from build123d import *

# Parameters (mm, degrees)
BOSS_EXTRUDE1_DEPTH = 580
BOSS_EXTRUDE2_DEPTH = 472
BOSS_EXTRUDE3_DEPTH = 580


with BuildPart() as part:
    # Sketch1 → Boss-Extrude1 (new body)
    with BuildSketch(Plane.XY):
        Polygon((-10.73531847, 12.748914521), (-45.73531847, 12.748914521), (-45.73531847, -37.251085479), (-10.73531847, -37.251085479), (-10.73531847, -33.251085479), (-41.73531847, -33.251085479), (-41.73531847, 8.748914521), (-10.73531847, 8.748914521), align=None)
    extrude(amount=BOSS_EXTRUDE1_DEPTH)

    # Sketch2 → Boss-Extrude2 (add)
    with BuildSketch(Plane(origin=(-41.73531847, 0, 0), x_dir=(0, 0, -1), z_dir=(1, 0, 0))):
        Polygon((-545, 12.748914521), (-580, 12.748914521), (-580, -37.251085479), (-545, -37.251085479), (-545, -33.251085479), (-576, -33.251085479), (-576, 8.748914521), (-545, 8.748914521), align=None)
        Polygon((-35, -33.251085479), (-35, -37.251085479), (0, -37.251085479), (0, 12.748914521), (-35, 12.748914521), (-35, 8.748914521), (-4, 8.748914521), (-4, -33.251085479), align=None)
    extrude(amount=BOSS_EXTRUDE2_DEPTH)

    # Sketch3 → Boss-Extrude3 (add)
    with BuildSketch(Plane.XY.offset(580)):
        Polygon((399.26468153, 12.748914521), (434.26468153, 12.748914521), (434.26468153, -37.251085479), (399.26468153, -37.251085479), (399.26468153, -33.251085479), (430.26468153, -33.251085479), (430.26468153, 8.748914521), (399.26468153, 8.748914521), align=None)
    extrude(amount=-BOSS_EXTRUDE3_DEPTH)


solid = part.part
Here's how the part is built. I have some questions about the finished solid (model axes, mm). A direction names the side the tool comes from. Coordinates: 2 decimals unless noted, no trailing zeros. Order: outer loops, then holes, each group sorted by start corner. A loop starts at its lowest first (then second) coordinate and runs counter-clockwise, first axis right, second up. Notation, with made-up numbers: M 27.25,-32 L 75.25,-32 A13 cw 75.25,-26 Z; hole C 55,68 d4. An arc over 180 degrees is marked long. Answer as CSV lines item,"result". Start each with the question number.
1. We'd pull the mould along Z, two halves only. Please class faces 3 (the flat face through (434.265, -12, 294)), 4 (the flat face through (-41.735, -13, 286)), 5 (the flat face through (191, -12, 580)): released by +Z, released by -Z, zero draft, split by the parting line, or undercut.
2. I need wall thicknesses on line 1 (X direction, y = -21.5, z = 184.5); line 2 (Z direction, x = 402, y = 5); line 3 (Y direction, x = -18.5, z = 464). Which ranges of each line are inside material? Lowest first, please. Write a range as [from, to].
3. On a 3-axis mill with a long thin cutter (end or side, diameter ignored), from which of +Z, -Z, +X, -X, +Y, -Y can I reach the whole of each face in a straight line? I mean faces 1 (the flat face through (191, -12, 4)), 2 (the flat face through (409, -37.251, 291)). Say none if no direction works.
4. I want a section at C-C, the plane y = -16.5. Write out the boundary of the cut face in (x, z), and give its area (3 significant figures).
5. I want a section at A-A, the plane z = 138.5. Write out the boundary of the cut face in (x, y), and give its area (3 significant figures).
6. I want a section at B-B, the plane x = 79. Write out the boundary of the cut face in (y, z).
Recorded:
1,face 3,"zero draft"
1,face 4,"undercut"
1,face 5,"released by +Z"
2,line 1,"x = [-45.74, -41.74], [430.26, 434.26]"
2,line 2,"z = [0, 4], [576, 580]"
2,line 3,"y = [-37.25, -33.25], [8.75, 12.75]"
3,face 1,"none"
3,face 2,"+Z, -Z, +X, -X, -Y"
4,outline,"M -45.74,0 L 434.26,0 L 434.26,580 L -45.74,580 Z; hole M -41.74,4 L 430.26,4 L 430.26,576 L -41.74,576 Z"
4,area,"8,420 mm2"
5,outline,"M -45.74,-37.25 L -10.74,-37.25 L -10.74,-33.25 L -41.74,-33.25 L -41.74,8.75 L -10.74,8.75 L -10.74,12.75 L -45.74,12.75 Z; M 399.26,-37.25 L 434.26,-37.25 L 434.26,12.75 L 399.26,12.75 L 399.26,8.75 L 430.26,8.75 L 430.26,-33.25 L 399.26,-33.25 Z"
5,area,"896 mm2"
6,outline,"M -37.25,0 L 12.75,0 L 12.75,35 L 8.75,35 L 8.75,4 L -33.25,4 L -33.25,35 L -37.25,35 Z; M -37.25,545 L -33.25,545 L -33.25,576 L 8.75,576 L 8.75,545 L 12.75,545 L 12.75,580 L -37.25,580 Z"
